```python
from build123d import *

# Parameters (mm, degrees)
SKETCH1_R      = 40
EXTRUDE1_DEPTH = 65
SKETCH2_R      = 35
EXTRUDE2_DEPTH = 202
EXTRUDE3_START = 85
SKETCH3_R      = 35
EXTRUDE3_DEPTH = 85
CHAMFER1_SIZE  = 3
EXTRUDE4_DEPTH = 7.5
SKETCH5_R      = 30
EXTRUDE5_DEPTH = 10
SKETCH7_R      = 25
EXTRUDE6_DEPTH = 83
EXTRUDE7_DEPTH = 10
CHAMFER2_SIZE  = 1


with BuildPart() as part:
    # Sketch1 → Extrude1 (new body)
    with BuildSketch(Plane(origin=(0, 0, 0), x_dir=(0, 0, -1), z_dir=(1, 0, 0))):
        Circle(SKETCH1_R)
    extrude(amount=EXTRUDE1_DEPTH)

    # Sketch2 → Extrude2 (add)
    with BuildSketch(Plane(origin=(65, 0, 0), x_dir=(0, 0, -1), z_dir=(1, 0, 0))):
        Circle(SKETCH2_R)
    extrude(amount=EXTRUDE2_DEPTH)

    # Sketch3 → Extrude3 (add)
    with BuildSketch(Plane.ZY.offset(EXTRUDE3_START)):
        with Locations(Location((0, 0, 0), (0, 0, 180))):
            Circle(SKETCH3_R)
    extrude(amount=-EXTRUDE3_DEPTH)

    # Chamfer1
    chamfer1_edges = [part.edges().sort_by_distance(p)[0] for p in [
        (-85, 0, 35),
    ]]
    chamfer(chamfer1_edges, length=CHAMFER1_SIZE)

    # Sketch4 → Extrude4 (cut)
    with BuildSketch(Plane(origin=(0, 27.5, 0), x_dir=(-1, 0, 0), z_dir=(0, 1, 0))):
        with BuildLine():
            Line((-80, 10), (-140, 10))
            ThreePointArc((-140, 10), (-150, 0), (-140, -10))
            Line((-140, -10), (-80, -10))
            ThreePointArc((-80, -10), (-70, 0), (-80, 10))
        make_face()
    extrude(amount=EXTRUDE4_DEPTH, mode=Mode.SUBTRACT)

    # Sketch5 → Extrude5 (add)
    with BuildSketch(Plane(origin=(267, 0, 0), x_dir=(0, 0, -1), z_dir=(1, 0, 0))):
        Circle(SKETCH5_R)
    extrude(amount=EXTRUDE5_DEPTH)

    # Sketch7 → Extrude6 (add)
    with BuildSketch(Plane(origin=(277, 0, 0), x_dir=(0, 0, -1), z_dir=(1, 0, 0))):
        Circle(SKETCH7_R)
    extrude(amount=EXTRUDE6_DEPTH)

    # Sketch8 → Extrude7 (cut)
    with BuildSketch(Plane(origin=(0, 19.5, 0), x_dir=(-1, 0, 0), z_dir=(0, 1, 0))):
        with BuildLine():
            Line((-292, 7), (-348, 7))
            ThreePointArc((-348, 7), (-355, 0), (-348, -7))
            Line((-348, -7), (-292, -7))
            ThreePointArc((-292, -7), (-285, 0), (-292, 7))
        make_face()
    extrude(amount=EXTRUDE7_DEPTH, mode=Mode.SUBTRACT)

    # Chamfer2
    chamfer2_edges = [part.edges().sort_by_distance(p)[0] for p in [
        (360, 0, 25),
    ]]
    chamfer(chamfer2_edges, length=CHAMFER2_SIZE)


solid = part.part
```
Geometry check sheet. Reference: the model listing, model coordinates, mm. A direction names the side the tool comes from. Give positions to 0.01 mm unless a question says otherwise; leave off trailing zeros. Order: outer loops, then holes, each group sorted by start corner. A loop starts at its lowest first (then second) coordinate and runs counter-clockwise, first axis right, second up. Notation, with made-up numbers: (-24, 53.5) - (-2, 53.5) arc R15 cw to (-2, 73.5) - close; hole circle Ø2 at (22, 33). An arc over 180 degrees is marked (long way). Answer in a Markdown table with one row per item. Add a question column.
Q1. Material ranges on probe 1 along Z at (x, y) = (235.5, 24.5) (3 decimals); probe 2 along Y at (x, z) = (142, -14); probe 3 along X at (y, z) = (-13, 28.5), recorded low to high. Write a range as from..to.
Q2. Cross-section at C-C, the plane x = 36.5. Enter the section's corners in (y, z), then the cut area to 3 significant figures.
Q3. Cross-section at A-A, the plane y = 0. Enter the section's corners in (x, z), then the cut area to 3 significant figures.
Q4. Cross-section at D-D, the plane x = 88.5. Enter the section's corners in (y, z), then the cut area to 3 significant figures.
Q5. Gauge pin test, flat ends, axial feed: pin 1 (1.3 mm diameter, centred on x = 318, y = 21.5, fed in from -Z); pin 2 (6 mm diameter, centred on x = 265, z = 1, fed in from -Y); pin 3 (12 mm diameter, centred on x = 158, z = -23.5, fed in from +Y). Record the tip position at first contact, or that the pin passes through.
Q6. Tool access check on faces 5 (the cylindrical face through (164.586, -34.168, 7.587)), 6 (the cylindrical face through (355, 22, 0)), 7 (the cylindrical face through (-41.574, 34.168, 7.587)). Record the directions out of +Z, -Z, +X, -X, +Y, -Y that give a thin tool (end or side, any length) a straight path to the whole face; none if there is none.
Q7. Mould release check, pull along Z, two halves, no side actions. Record for faces 1 (the flat face through (360, 0, 0)), 2 (the cylindrical face through (70, 31, 0)), 3 (the cylindrical face through (150, 31, 0)), 4 (the cylindrical face through (271.93, 1.32, 29.97)): pulls with the +Z half, pulls with the -Z half, needs draft (parallel to the pull), parting line crosses it, or undercut.
Check values:
| question | item | result |
|---|---|---|
| 1 | probe 1 | z = -24.995..24.995 |
| 1 | probe 2 | y = -32.08..32.08 |
| 1 | probe 3 | x = -85..267 |
| 2 | outline | circle Ø80 at (0, 0) |
| 2 | area | 5,030 mm^2 |
| 3 | outline | (-85, -32) - (-82, -35) - (0, -35) - (0, -40) - (65, -40) - (65, -35) - (267, -35) - (267, -30) - (277, -30) - (277, -25) - (359, -25) - (360, -24) - (360, 24) - (359, 25) - (277, 25) - (277, 30) - (267, 30) - (267, 35) - (65, 35) - (65, 40) - (0, 40) - (0, 35) - (-82, 35) - (-85, 32) - close |
| 3 | area | 30,000 mm^2 |
| 4 | outline | (27.5, -10) - (27.5, 10) - (33.54, 10) arc R35 ccw (long way) to (33.54, -10) - close |
| 4 | area | 3,710 mm^2 |
| 5 | pin 1 | stops at z = -13.79 |
| 5 | pin 2 | stops at y = -35 |
| 5 | pin 3 | stops at y = 30.31 |
| 6 | face 5 | +X |
| 6 | face 6 | +Y |
| 6 | face 7 | -X |
| 7 | face 1 | needs draft |
| 7 | face 2 | undercut |
| 7 | face 3 | undercut |
| 7 | face 4 | parting line crosses it |
